from build123d import *

# Parameters (mm, degrees)
EXTRUDE_1_DEPTH     = 456
CUT_EXTRUDE_1_DEPTH = 40


with BuildPart() as part:
    # 草图1 → 拉伸1 (new body)
    with BuildSketch(Plane.XY):
        with BuildLine():
            Line((0, 0), (0, 40))
            Line((0, 40), (3.99, 40))
            ThreePointArc((3.99, 40), (3.997071068, 39.997071068), (4, 39.99))
            Line((4, 39.99), (4, 9))
            ThreePointArc((4, 9), (5.464466094, 5.464466094), (9, 4))
            Line((9, 4), (39.99, 4))
            ThreePointArc((39.99, 4), (39.997071068, 3.997071068), (40, 3.99))
            Line((40, 3.99), (40, 0))
            Line((40, 0), (0, 0))
        make_face()
    extrude(amount=EXTRUDE_1_DEPTH)

    # 草图2 → 切除-拉伸1 (cut)
    with BuildSketch(Plane(origin=(0, 40, 0), x_dir=(1, 0, 0), z_dir=(0, 1, 0))):
        Polygon((5, -456), (0, -451), (0, -456), align=None)
        Polygon((0, 0), (0, -5), (5, 0), align=None)
    extrude(amount=-CUT_EXTRUDE_1_DEPTH, mode=Mode.SUBTRACT)


solid = part.part
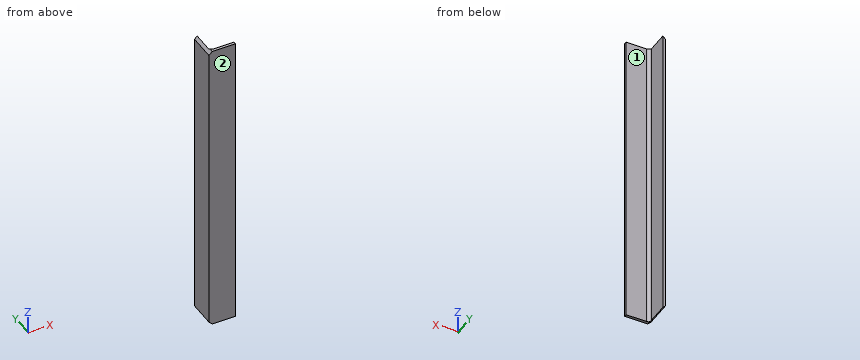
Check sheet for the modelled part. Datum: model origin and axes. Units: mm. Face numbers are marked on the shaded views. A direction names the side the tool comes from. Coordinates: 2 decimals unless noted, no trailing zeros. Write each loop counter-clockwise with the first axis right and the second up, starting at its lowest first coordinate (ties: lowest second). Pieces come first, ordered by that corner, then holes.
Item 1: Scan lines: probe 1 along X at (y, z) = (10, 322.5); probe 2 along X at (y, z) = (6, 200). Record each from-to range of solid material in increasing order.
Numbers:
probe 1: x = 0 to 4
probe 2: x = 0 to 5
Item 2: Cross-section at C-C on x = 23. Record the boundary of the cut face in (y, z), then the cut area to 3 significant figures.
Numbers:
outline: (0, 0) - (4, 0) - (4, 456) - (0, 456) - close
area: 1,820 mm2
Item 3: Cross-section at B-B on y = 32. Record the boundary of the cut face in (x, z).
Numbers:
outline: (0, 5) - (4, 1) - (4, 455) - (0, 451) - close
Item 4: Depth check by flat-ended pin: pin 1 Ø10 at (x, z) = (35.5, 122.5) entering from +Y; pin 2 Ø3 at (x, y) = (26.5, 4.5) entering from -Z; pin 3 Ø6 at (x, y) = (5, 11) entering from +Z; pin 4 Ø15.5 at (y, z) = (24, 166.5) entering from +X. Enter the tip coordinate at first touch or a pass-through.
Numbers:
pin 1: stops at y = 4
pin 2: stops at z = 0
pin 3: stops at z = 455.07
pin 4: stops at x = 4
Item 5: Access from +Z, -Z, +X, -X, +Y, -Y to the whole of each face (thin tool, end or side, straight path). Record for the marked faces 1 and 2.
Numbers:
face 1: +Z, -Z, +X, +Y
face 2: +Z, -Z, +X, -X, -Y
